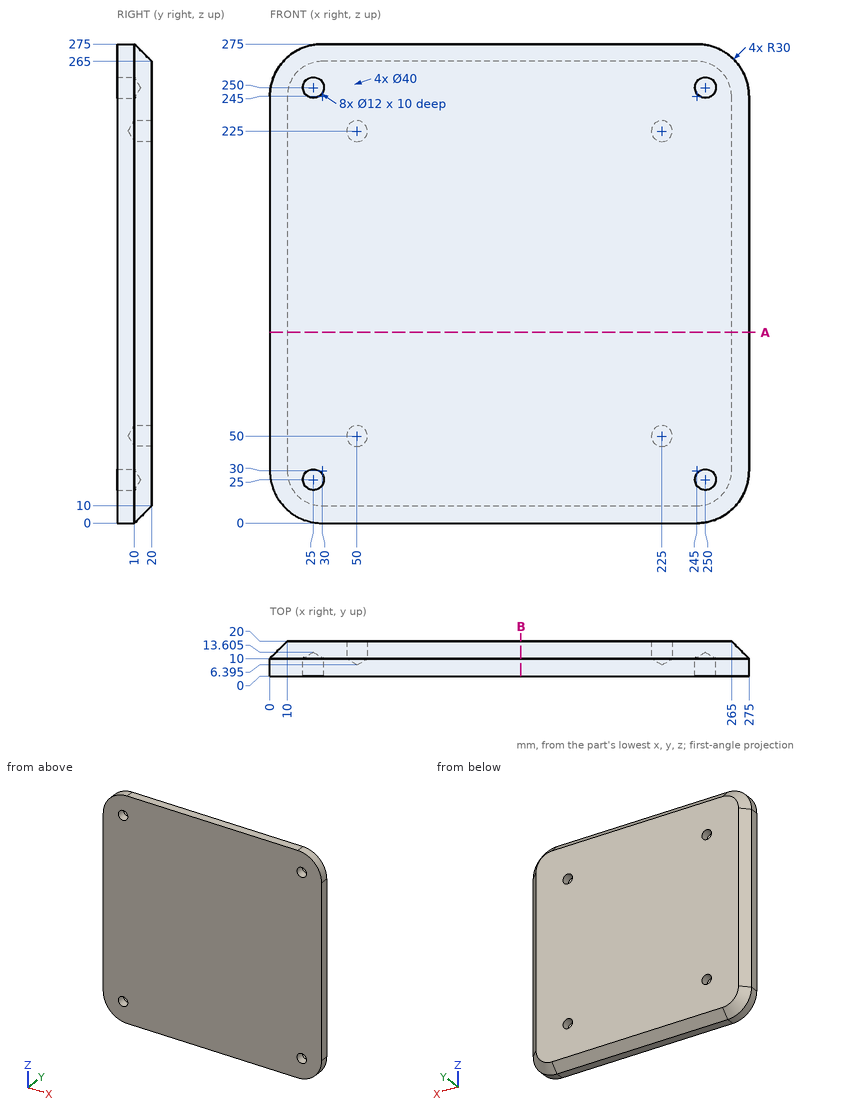
Study the drawing (mm; zero at the part's minimum x, y, z) and answer. Coordinates: 2 decimals unless noted, no trailing zeros. Write each loop counter-clockwise with the first axis right and the second up, starting at its lowest first coordinate (ties: lowest second). Pieces come first, ordered by that corner, then holes. Notation, with made-up numbers: (-34.5, 19) - (17.5, 19) arc R4 cw to (17.5, 24) - close; hole circle Ø10 at (-14, 8). An arc over 180 degrees is marked (long way). Put each result on its own line as item: value.
1. Find the intervals of material crossed by line 1 along X through (y, z) = (6.5, 250); line 2 along Z through (x, y) = (225, 14.75), in increasing order. Write a range as from..to.
Answer sheet:
line 1: x = 0.42..19, 31..244, 256..274.58
line 2: z = 4.75..44, 56..219, 231..270.25
2. A flat-ended cylindrical pin translates along its axis: pin 1 Ø6 at (y, z) = (17.5, 196.5) entering from +X. Find the tip coordinate at first contact, or state that the pin passes through.
Answer sheet:
pin 1: stops at x = 270.5
3. The part is cut by section B-B on x = 144. Give the vertices of the cut face in (y, z).
Answer sheet:
outline: (0, 0) - (10, 0) - (20, 10) - (20, 265) - (10, 275) - (0, 275) - close
4. The part is cut by section A-A on z = 109.5. Give the vertices of the cut face in (x, y).
Answer sheet:
outline: (0, 0) - (275, 0) - (275, 10) - (265, 20) - (10, 20) - (0, 10) - close
